CAD build for the part. Positions are in the model's coordinates, mm. A direction names the side the tool comes from. Round coordinates to 2 decimals unless told otherwise and drop trailing zeros. Order: outer loops, then holes, each group sorted by start corner. A loop starts at its lowest first (then second) coordinate and runs counter-clockwise, first axis right, second up.
```python
from build123d import *

# Parameters (mm, degrees)
SKETCH1_R           = 8
SKETCH1_R_2         = 6.6
BOSS_EXTRUDE1_DEPTH = 7
SKETCH2_W           = 5.5
SKETCH2_H           = 7.166353003
CUT_EXTRUDE1_DEPTH  = 14.304134696
CHAMFER1_SIZE       = 0.5


with BuildPart() as part:
    # Sketch1 → Boss-Extrude1 (new body)
    with BuildSketch(Plane.XY):
        Circle(SKETCH1_R)
        Circle(SKETCH1_R_2, mode=Mode.SUBTRACT)
    extrude(amount=BOSS_EXTRUDE1_DEPTH)

    # Sketch2 → Cut-Extrude1 (cut, through all)
    with BuildSketch(Plane.XY.offset(7)):
        with Locations((0, 7.454286829)):
            Rectangle(SKETCH2_W, SKETCH2_H)
    extrude(amount=-CUT_EXTRUDE1_DEPTH, mode=Mode.SUBTRACT)

    # Chamfer1
    chamfer1_edges = [part.edges().sort_by_distance(p)[0] for p in [
        (0, -6.6, 0),
        (0, -6.6, 7),
    ]]
    chamfer(chamfer1_edges, length=CHAMFER1_SIZE)


solid = part.part
```
1. Cut at A-A, the plane y = 0. Write the cut outline in (x, z), and give its area (3 significant figures).
2. Cut at C-C, the plane z = 3.5. Write the cut outline in (x, y), and give its area (3 significant figures).
3. Cut at B-B, the plane x = 0. Write the cut outline in (y, z).
4. Pin check, flat tips, straight feed: P1, Ø0.5, axis at y = 7, z = 4.5, coming from the -X side; P2, Ø1, axis at y = 4, z = 4, coming from the +X side; P3, Ø1.5, axis at x = -5.5, z = 1.5, coming from the +Y side; P4, Ø1.5, axis at x = -5.5, y = -4, coming from the -Z side. Stop position of each tip, or through.
5. Mould opens along Y. For faces 1 (the face through (0.259, -6.737, 6.642)), 2 (the face through (0, -8, 3)), 3 (the face through (-2.75, 7, 4)) say: released by +Y, released by -Y, zero draft, split by the parting line, or undercut.
6. Tool access for faces 4 (the face through (-0.251, -6.595, 3.458)), 5 (the face through (2.75, 7, 4)): list every direction of +Z, -Z, +X, -X, +Y, -Y with a clear straight run to the whole face (end or side of a thin tool).
7. Drill centre lines: line 1 (X direction, y = 0, z = 2.65); line 2 (Y direction, x = -3, z = 6.75); line 3 (X direction, y = -5.5, z = 5.75). Where is each one in solid material? Low to high.
Outcome:
1. outline: (-8, 0) - (-7.1, 0) - (-6.6, 0.5) - (-6.6, 6.5) - (-7.1, 7) - (-8, 7) - close; (6.6, 0.5) - (7.1, 0) - (8, 0) - (8, 7) - (7.1, 7) - (6.6, 6.5) - close
1. area: 19.1 mm2
2. outline: (-2.75, 6) - (-2.75, 7.51) arc R8 ccw (long way) to (2.75, 7.51) - (2.75, 6) arc R6.6 cw (long way) to start
2. area: 56.3 mm2
3. outline: (-8, 0) - (-7.1, 0) - (-6.6, 0.5) - (-6.6, 6.5) - (-7.1, 7) - (-8, 7) - close
4. P1: stops at x = -4.29
4. P2: stops at x = 7.19
4. P3: stops at y = 6.44
4. P4: stops at z = 0
5. face 1: undercut
5. face 2: split by the parting line
5. face 3: zero draft
6. face 4: +Z, -Z
6. face 5: +Z, -Z, +Y
7. line 1: x = -8 to -6.6, 6.6 to 8
7. line 2: y = -7.42 to -6.16, 6.16 to 7.42
7. line 3: x = -5.81 to -3.65, 3.65 to 5.81
